```python
from build123d import *

# Parameters (mm, degrees)
BASE_BLOCK_DEPTH           = 60
ARM_DEPTH                  = 60
ARM_TRIM_CUT_DEPTH         = 45
HUB_SKETCH_32_R            = 16
HUB_32_DEPTH               = 20
HUB_START                  = 15
HUB_EXTENSION_SKETCH_32_R  = 16
HUB_EXTENSION_32_DEPTH     = 15
BORE_SKETCH_22_R           = 11
HUB_BORE_22_DEPTH          = 40
MOUNTING_HOLES_SKETCH_R    = 8.5
MOUNTING_HOLES_2X_17_DEPTH = 18


with BuildPart() as part:
    # Base Profile Sketch → Base Block (new body)
    with BuildSketch(Plane.XY):
        Polygon((0, 0), (-75, 0), (-75, -30), (-55, -30), (-55, -18), (0, -18), align=None)
    extrude(amount=BASE_BLOCK_DEPTH)

    # Arm Profile Sketch → Arm (add)
    with BuildSketch(Plane(origin=(0, 0, 0), x_dir=(-1, 0, 0), z_dir=(0, 0, -1))):
        Polygon((0, 0), (75, 0), (140, 58), (140, 73), (95, 40), align=None)
    extrude(amount=-ARM_DEPTH)

    # Arm Trim Sketch → Arm Trim Cut (cut)
    with BuildSketch(Plane(origin=(0, 0, 0), x_dir=(-1, 0, 0), z_dir=(0, 0, -1))):
        Polygon((0, 0), (95, 40), (140, 73), (140, 58), (75, 0), align=None)
    extrude(amount=-ARM_TRIM_CUT_DEPTH, mode=Mode.SUBTRACT)

    # Hub Sketch Ø32 → Hub Ø32 (add)
    with BuildSketch(Plane(origin=(0, 0, 45), x_dir=(-1, 0, 0), z_dir=(0, 0, -1))):
        with Locations((140, 65.5)):
            Circle(HUB_SKETCH_32_R)
    extrude(amount=-HUB_32_DEPTH)

    # Hub Extension Sketch Ø32 → Hub Extension Ø32 (add)
    with BuildSketch(Plane(origin=(0, 0, 45), x_dir=(-1, 0, 0), z_dir=(0, 0, -1)).offset(HUB_START)):
        with Locations((140, 65.5)):
            Circle(HUB_EXTENSION_SKETCH_32_R)
    extrude(amount=-HUB_EXTENSION_32_DEPTH)

    # Bore Sketch Ø22 → Hub Bore Ø22 (cut)
    with BuildSketch(Plane(origin=(0, 0, 30), x_dir=(-1, 0, 0), z_dir=(0, 0, -1))):
        with Locations((140, 65.5)):
            Circle(BORE_SKETCH_22_R)
    extrude(amount=-HUB_BORE_22_DEPTH, mode=Mode.SUBTRACT)

    # Mounting Holes Sketch → Mounting Holes 2xØ17 (cut)
    with BuildSketch(Plane(origin=(0, 0, 0), x_dir=(1, 0, 0), z_dir=(0, 1, 0))):
        with Locations(Location((-12, -25, 0), (0, 0, 270))):
            Circle(MOUNTING_HOLES_SKETCH_R)
        with Locations(Location((-37, -25, 0), (0, 0, 270))):
            Circle(MOUNTING_HOLES_SKETCH_R)
    extrude(amount=-MOUNTING_HOLES_2X_17_DEPTH, mode=Mode.SUBTRACT)


solid = part.part
```
Here's how the part is built. I have some questions about the finished solid (model axes, mm). A direction names the side the tool comes from. Give positions to 0.01 mm unless a question says otherwise; leave off trailing zeros. Order: outer loops, then holes, each group sorted by start corner. A loop starts at its lowest first (then second) coordinate and runs counter-clockwise, first axis right, second up. Notation, with made-up numbers: (1.5, 62) - (12.5, 62) arc R27 ccw to (12.5, 92) - close; hole circle Ø10 at (37.25, -10). An arc over 180 degrees is marked (long way). Answer as a JSON object with one key per item and string values. Group by question number.
Item 1: If we section it at A-A on y = 65.5: Please give me the cut outline in (x, z), and give its area (3 significant figures).
Item 2: If we section it at B-B on z = 21: Please give me the cut outline in (x, y).
Item 3: Which directions (+Z, -Z, +X, -X, +Y, -Y) give clear straight access to the entire face, cutting with the end or side of a thin tool? Please do faces 1 (the flat face through (-136, 55, 30)), 2 (the flat face through (-28, -18, 30)), 3 (the flat face through (-46, 0, 22)), 4 (the cylindrical face through (-129.01, 65.98, 47.26)), 5 (the flat face through (-75, -15, 30)).
Item 4: If we section it at C-C on x = -140: Please give me the cut outline in (y, z).
Item 5: For P1, Ø4, axis at x = -64, z = 39.5, coming from the +Y side; P2, Ø15, axis at y = -13, z = 36.5, coming from the -X side; P3, Ø18.5, axis at x = -65, y = 34, coming from the -Z side, each with a flat end and sliding along its axis, tell me the tip position at first contact or that it passes through.
Item 6: If we mould it in two halves opening along Z, with no side actions, what happens to faces 6 (the flat face through (-76, 20, 45)), 7 (the cylindrical face through (-4.833, -8.874, 29.57)), 8 (the cylindrical face through (-45.3, -8.87, 23.16)), 9 (the flat face through (-65, -30, 30))? For each: pulls with the +Z half, pulls with the -Z half, needs draft (parallel to the pull), parting line crosses it, or undercut.
Item 7: Please list where these lines run through material, in increasing order: probe 1 along X at (y, z) = (-3.25, 25); probe 2 along Y at (x, z) = (-140, 52); probe 3 along Y at (x, z) = (-13, 3).
Item 8: If we section it at D-D on y = -3.5: Please give me the cut outline in (x, z), and give its area (3 significant figures).
Result set:
{
 "1": {"outline": "(-156, 30) - (-151, 30) - (-151, 65) - (-156, 65) - close; (-129, 30) - (-124, 30) - (-124, 65) - (-129, 65) - close", "area": "350 mm²"},
 "2": {"outline": "(-75, -30) - (-55, -30) - (-55, -18) - (-44.5, -18) - (-44.5, 0) - (-75, 0) - close; (-29.5, -18) - (-19.5, -18) - (-19.5, 0) - (-29.5, 0) - close; (-4.5, -18) - (0, -18) - (0, 0) - (-4.5, 0) - close"},
 "3": {"face 1": "-Z, +X, -X, +Y, -Y", "face 2": "+Z, -Z, +X, -Y", "face 3": "-Z, +X, -X, +Y", "face 4": "+Z, -Z", "face 5": "+Z, -Z, -X, -Y"},
 "4": {"outline": "(49.5, 30) - (54.5, 30) - (54.5, 65) - (49.5, 65) - close; (76.5, 30) - (81.5, 30) - (81.5, 65) - (76.5, 65) - close"},
 "5": {"P1": "y = 0", "P2": "x = -75", "P3": "z = 45"},
 "6": {"face 6": "pulls with the -Z half", "face 7": "undercut", "face 8": "undercut", "face 9": "needs draft"},
 "7": {"probe 1": "-75 to -45.5, -28.5 to -20.5, -3.5 to 0", "probe 2": "49.5 to 54.5, 76.5 to 81.5", "probe 3": "-18 to 0"},
 "8": {"outline": "(-75, 0) - (0, 0) - (0, 60) - (-75, 60) - close; hole circle Ø17 at (-37, 25); hole circle Ø17 at (-12, 25)", "area": "4,050 mm²"}
}
